```python
from build123d import *

# Parameters (mm, degrees)
EXTRUDE_1_DEPTH = 2
FILLET_1_R      = 3


with BuildPart() as part:
    # 草图1 → 凸台-拉伸1 (new body)
    with BuildSketch(Plane.XY):
        with BuildLine():
            Line((-7, 106.65), (-7, -106.65))
            Line((-7, -106.65), (-10.1, -112.75))
            Line((-10.1, -112.75), (-10.1, -118.75))
            Line((-10.1, -118.75), (-7.1, -118.75))
            Line((-7.1, -118.75), (-7.1, -113.75))
            ThreePointArc((-7.1, -113.75), (0, -106.65), (7.1, -113.75))
            Line((7.1, -113.75), (7.1, -118.75))
            Line((7.1, -118.75), (10.1, -118.75))
            Line((10.1, -118.75), (10.1, -112.75))
            Line((10.1, -112.75), (7, -106.65))
            Line((7, -106.65), (7, 106.65))
            Line((7, 106.65), (10.1, 112.75))
            Line((10.1, 112.75), (10.1, 118.75))
            Line((10.1, 118.75), (7.1, 118.75))
            Line((7.1, 118.75), (7.1, 113.75))
            ThreePointArc((7.1, 113.75), (0, 106.65), (-7.1, 113.75))
            Line((-7.1, 113.75), (-7.1, 118.75))
            Line((-7.1, 118.75), (-10.1, 118.75))
            Line((-10.1, 118.75), (-10.1, 112.75))
            Line((-10.1, 112.75), (-7, 106.65))
        make_face()
        with BuildLine():
            Line((3, 98), (3, 42))
            ThreePointArc((3, 42), (0, 39), (-3, 42))
            Line((-3, 42), (-3, 98))
            ThreePointArc((-3, 98), (0, 101), (3, 98))
        make_face(mode=Mode.SUBTRACT)
        with BuildLine():
            Line((3, 28), (3, -28))
            ThreePointArc((3, -28), (0, -31), (-3, -28))
            Line((-3, -28), (-3, 28))
            ThreePointArc((-3, 28), (0, 31), (3, 28))
        make_face(mode=Mode.SUBTRACT)
        with BuildLine():
            Line((3, -40), (3, -90))
            ThreePointArc((3, -90), (0, -93), (-3, -90))
            Line((-3, -90), (-3, -40))
            ThreePointArc((-3, -40), (0, -37), (3, -40))
        make_face(mode=Mode.SUBTRACT)
    extrude(amount=EXTRUDE_1_DEPTH)

    # 圆角1
    fillet_1_edges = [part.edges().sort_by_distance(p)[0] for p in [
        (10.1, 112.75, 1),
        (7, 106.65, 1),
        (7, -106.65, 1),
        (10.1, -112.75, 1),
        (-10.1, -112.75, 1),
        (-7, -106.65, 1),
        (-7, 106.65, 1),
        (-10.1, 112.75, 1),
    ]]
    fillet(fillet_1_edges, radius=FILLET_1_R)


solid = part.part
```
Could you check a few things on this model? Use its own coordinates, in mm. Coordinates: 2 decimals unless noted, no trailing zeros. Order: outer loops, then holes, each group sorted by start corner. A loop starts at its lowest first (then second) coordinate and runs counter-clockwise, first axis right, second up. Notation, with made-up numbers: M 80,-7 L 118,-7 A31 ccw 118,22 Z; hole C 47.5,-25.75 d9. An arc over 180 degrees is marked long. Use one line per item in the form item = value. Start each with the question number.
1. We'd pull the mould along X, two halves only. Please class faces 1 (the cylindrical face through (-0.16, -106.65, 0.99)), 2 (the flat face through (-5, 2, 2)): +X half, -X half, draft (parallel to the pull), parting line (faces both ways), or undercut.
2. Please list where these lines run through material, in increasing order: line 1 (Y direction, x = -0.5, z = 1.6); line 2 (X direction, y = 6, z = 1.35); line 3 (Y direction, x = 1, z = 0.4).
3. For pin 1 (1 mm diameter, centred on y = -5, z = 0.5, fed in from +X); pin 2 (0.6 mm diameter, centred on y = 3, z = 1, fed in from -X), each with a flat end and sliding along its axis, tell me the tip position at first contact or that it passes through.
4. Suppose I cut it at C-C on z = 0.8. Count the separate pieces of the cut face and the enclosed holes in it, then the cut area to 3 significant figures.
5. Suppose I cut it at A-A on y = -56. Write out the boundary of the cut face in (x, z).
6. Suppose I cut it at B-B on x = 0. Write out the boundary of the cut face in (y, z).
Geometry says:
q1.face_1 = undercut
q1.face_2 = draft
q2.line_1 = -106.67 to -92.96, -37.04 to -30.96, 30.96 to 39.04, 100.96 to 106.67
q2.line_2 = -7 to -3, 3 to 7
q2.line_3 = -106.72 to -92.83, -37.17 to -30.83, 30.83 to 39.17, 100.83 to 106.72
q3.pin_1 = 7
q3.pin_2 = -7
q4.separate_pieces = 1
q4.enclosed_holes = 3
q4.area = 2,080 mm^2
q5.outline = M -7,0 L -3,0 L -3,2 L -7,2 Z; M 3,0 L 7,0 L 7,2 L 3,2 Z
q6.outline = M -106.65,0 L -93,0 L -93,2 L -106.65,2 Z; M -37,0 L -31,0 L -31,2 L -37,2 Z; M 31,0 L 39,0 L 39,2 L 31,2 Z; M 101,0 L 106.65,0 L 106.65,2 L 101,2 Z
